Check sheet for the drawn part. Datum: minimum x, y, z corner. Units: mm. A direction names the side the tool comes from. Coordinates: 2 decimals unless noted, no trailing zeros. Loops run counter-clockwise (first coordinate to the right, second up) from the corner with the lowest first, then second, coordinate; pieces in that order, holes last. Notation, with made-up numbers: (0, 6.25) -> (6, 6.25) arc R11 ccw to (6, 18.25) -> close; hole circle Ø5 at (54.5, 44.25). An arc over 180 degrees is marked (long way). Use CSV: the item, a comma, the result in double quotes. Start each with the question number.
1. Thickness scan on L1, parallel to X at y = 12.1, z = 25.75; L2, parallel to Y at x = 26, z = 8; L3, parallel to X at y = 10.75, z = 4.5. Record the ranges inside material, lowest first.
2. Sectioned sample at A-A, the plane x = 25.75. Record the cut outline in (y, z), and give its area (4 significant figures).
3. Sectioned sample at B-B, the plane z = 3.75. Record the cut outline in (x, y).
4. Sectioned sample at D-D, the plane x = 14.75. Record the cut outline in (y, z).
5. Release check for a two-part mould opening along X. For the marked faces 1, 2, 3 and 4 record: pulls with the +X half, pulls with the -X half, needs draft (parallel to the pull), parting line crosses it, or undercut.
6. Sectioned sample at C-C, the plane z = 14.75. Record the cut outline in (x, y).
7. Gauge pin test, flat ends, axial feed: pin 1 (8.5 mm diameter, centred on x = 17, z = 16, fed in from +Y); pin 2 (2 mm diameter, centred on y = 8, z = 13.5, fed in from +X); pin 3 (4 mm diameter, centred on y = 2, z = 22.5, fed in from +X); pin 4 (2.5 mm diameter, centred on x = 25.75, z = 3.75, fed in from +Y). Record the tip position at first contact, or that the pin passes through.
8. Set-up check for the marked faces 5, 6 and 7: record each of +Z, -Z, +X, -X, +Y, -Y from which the full face is reachable in a straight line by a thin tool's end or side.
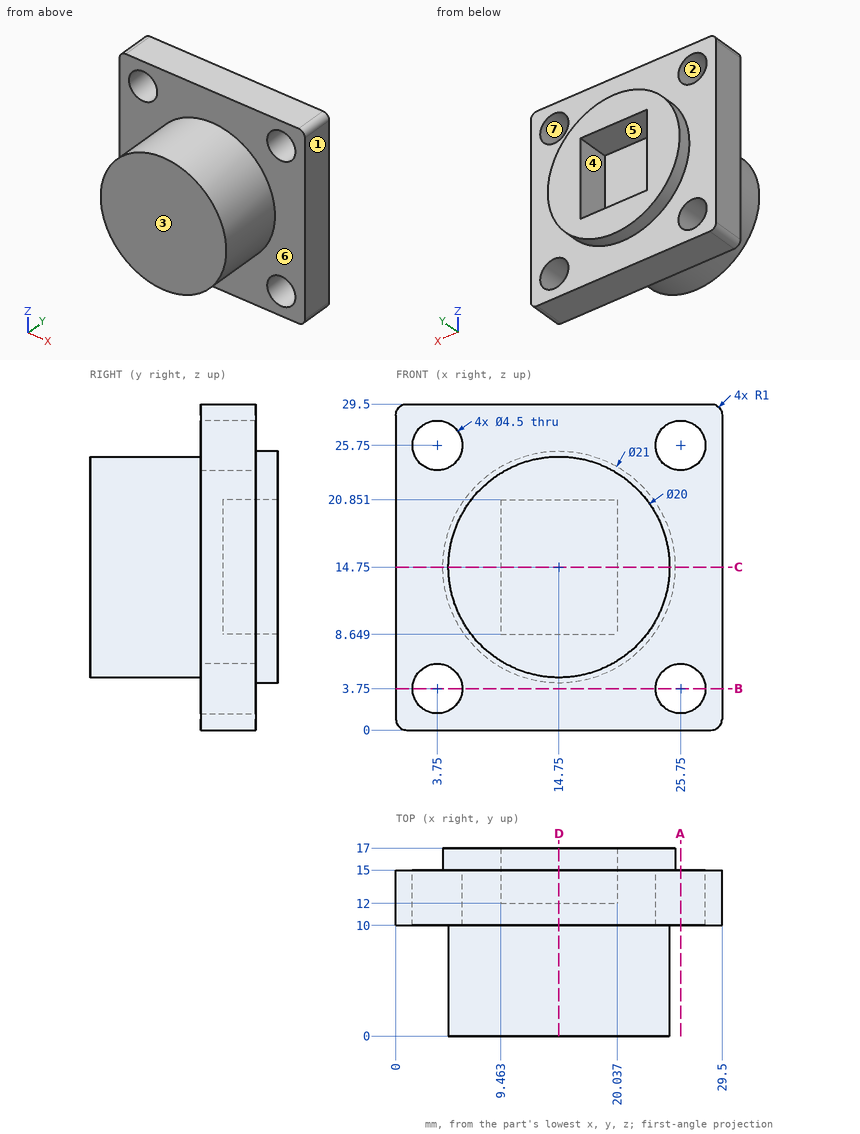
Completed:
1,L1,"0 to 1.5, 6 to 23.5, 28 to 29.5"
1,L2,"10 to 15"
1,L3,"0 to 1.63, 5.87 to 23.63, 27.87 to 29.5"
2,outline,"(10, 0) -> (15, 0) -> (15, 1.5) -> (10, 1.5) -> close; (10, 6) -> (15, 6) -> (15, 23.5) -> (10, 23.5) -> close; (10, 28) -> (15, 28) -> (15, 29.5) -> (10, 29.5) -> close"
2,area,"102.5 mm²"
3,outline,"(0, 10) -> (1.5, 10) -> (1.5, 15) -> (0, 15) -> close; (6, 10) -> (23.5, 10) -> (23.5, 15) -> (6, 15) -> close; (28, 10) -> (29.5, 10) -> (29.5, 15) -> (28, 15) -> close"
4,outline,"(0, 4.75) -> (10, 4.75) -> (10, 0) -> (15, 0) -> (15, 4.25) -> (17, 4.25) -> (17, 8.65) -> (12, 8.65) -> (12, 20.85) -> (17, 20.85) -> (17, 25.25) -> (15, 25.25) -> (15, 29.5) -> (10, 29.5) -> (10, 24.75) -> (0, 24.75) -> close"
5,face 1,"pulls with the +X half"
5,face 2,"undercut"
5,face 3,"needs draft"
5,face 4,"undercut"
6,outline,"(0, 10) -> (4.75, 10) -> (4.75, 0) -> (24.75, 0) -> (24.75, 10) -> (29.5, 10) -> (29.5, 15) -> (25.25, 15) -> (25.25, 17) -> (20.04, 17) -> (20.04, 12) -> (9.46, 12) -> (9.46, 17) -> (4.25, 17) -> (4.25, 15) -> (0, 15) -> close"
7,pin 1,"y = 17"
7,pin 2,"x = 24.75"
7,pin 3,"x = 22.93"
7,pin 4,"through"
8,face 5,"+Y"
8,face 6,"-Y"
8,face 7,"+Y, -Y"
